Can you work these out from the model? Positions are in its coordinate system, mm. A direction names the side the tool comes from. Round coordinates to 2 decimals unless told otherwise and drop trailing zeros. Loops run counter-clockwise (first coordinate to the right, second up) from the corner with the lowest first, then second, coordinate; pieces in that order, holes last. Notation, with made-up numbers: (-1.75, 3.25) -> (39.25, 3.25) arc R29 ccw to (39.25, 38.25) -> close; hole circle Ø9 at (-40, -21.75). An arc over 180 degrees is marked (long way). Answer as a JSON object with one key per item and string values.
```python
from build123d import *

# Parameters (mm, degrees)
SKETCH1_W                                            = 2260
SKETCH1_H                                            = 50
BOSS_EXTRUDE1_DEPTH                                  = 5
BOSS_EXTRUDE2_DEPTH                                  = 2260
CSK_FOR_M6_HEXAGON_LOBULAR_SOCKET_RAISED_D           = 6.6
CSK_FOR_M6_HEXAGON_LOBULAR_SOCKET_RAISED_DEPTH       = 19.75
CSK_FOR_M6_HEXAGON_LOBULAR_SOCKET_RAISED_CSINK_D     = 12.8
CSK_FOR_M6_HEXAGON_LOBULAR_SOCKET_RAISED_CSINK_ANGLE = 90
CSK_FOR_M6_HEXAGON_LOBULAR_SOCKET_RAISED_TIP         = 1.982840043


with BuildPart() as part:
    # Sketch1 → Boss-Extrude1 (new body)
    with BuildSketch(Plane.XY):
        Rectangle(SKETCH1_W, SKETCH1_H)
    extrude(amount=BOSS_EXTRUDE1_DEPTH)

    # Sketch2 → Boss-Extrude2 (add)
    with BuildSketch(Plane.ZY.offset(1130)):
        Polygon((0, 25), (-22, 25), (-35, 20.5), (-35, 20), (0, 20), align=None)
    extrude(amount=-BOSS_EXTRUDE2_DEPTH)

    # CSK for M6 Hexagon lobular socket raised CTSK head screws1
    with Locations(Plane.XY.offset(5)):
        with Locations((-589, -11.306794409), (-559, -11.306794409), (-15, -11.306794409), (15, -11.306794409), (559, -11.306794409), (589, -11.306794409), (-1124, -12.5), (-1124, 12.5), (1124, -12.5), (1124, 12.5)):
            CounterSinkHole(CSK_FOR_M6_HEXAGON_LOBULAR_SOCKET_RAISED_D / 2, CSK_FOR_M6_HEXAGON_LOBULAR_SOCKET_RAISED_CSINK_D / 2, depth=CSK_FOR_M6_HEXAGON_LOBULAR_SOCKET_RAISED_DEPTH, counter_sink_angle=CSK_FOR_M6_HEXAGON_LOBULAR_SOCKET_RAISED_CSINK_ANGLE)
            with Locations((0, 0, -(CSK_FOR_M6_HEXAGON_LOBULAR_SOCKET_RAISED_DEPTH + CSK_FOR_M6_HEXAGON_LOBULAR_SOCKET_RAISED_TIP / 2))):  # 118° drill point
                Cone(0, CSK_FOR_M6_HEXAGON_LOBULAR_SOCKET_RAISED_D / 2, CSK_FOR_M6_HEXAGON_LOBULAR_SOCKET_RAISED_TIP, mode=Mode.SUBTRACT)


solid = part.part
```
Q1. On a 3-axis mill with a long thin cutter (end or side, diameter ignored), from which of +Z, -Z, +X, -X, +Y, -Y can I reach the whole of each face in a straight line? I mean faces 1 (the flat face through (-16, 20, -18)), 2 (the flat face through (-1130, 9, 1)). Say none if no direction works.
Determined:
{"face 1": "-Z, +X, -X, -Y", "face 2": "+Z, -Z, -X, +Y, -Y"}
Q2. I'm going to push flat-ended pins straight in: pin 1 (6 mm diameter, centred on x = -567.5, y = 3, fed in from -Z); pin 2 (7.5 mm diameter, centred on x = 15, y = -11.31, fed in from +Z); pin 3 (5.5 mm diameter, centred on x = -559, y = -11.31, fed in from -Z); pin 4 (8.5 mm diameter, centred on x = 1124, y = -12.5, fed in from +Z). Where does each tip first touch, or does it pass through?
Determined:
{"pin 1": "z = 0", "pin 2": "z = 2.35", "pin 3": "through", "pin 4": "z = 2.85"}
Q3. I want a section at B-B, the plane z = -9.5. Write out the boundary of the cut face in (x, y), then the cut area to 3 significant figures.
Determined:
{"outline": "(-1130, 20) -> (1130, 20) -> (1130, 25) -> (-1130, 25) -> close", "area": "11,300 mm²"}
Q4. I want a section at A-A, the plane x = -279. Write out the boundary of the cut face in (y, z).
Determined:
{"outline": "(-25, 0) -> (20, 0) -> (20, -35) -> (20.5, -35) -> (25, -22) -> (25, 5) -> (-25, 5) -> close"}
Q5. If I drill on L1, parallel to X at y = 12.5, z = 1; L2, parallel to Y at x = -589, z = 1; L3, parallel to Y at x = 1124, z = 1.3, over which ranges is the centre line in solid material (lowest first)? Write a range as [from, to].
Determined:
{"L1": "[-1130, -1127.3], [-1120.7, 1120.7], [1127.3, 1130]", "L2": "[-25, -14.61], [-8.01, 25]", "L3": "[-25, -15.8], [-9.2, 9.2], [15.8, 25]"}
